Part print with two shaded views. Sizes in mm from the minimum x, y, z corner. A direction names the side the tool comes from. Round coordinates to 2 decimals unless told otherwise and drop trailing zeros. Loops run counter-clockwise (first coordinate to the right, second up) from the corner with the lowest first, then second, coordinate; pieces in that order, holes last. Notation, with made-up numbers: (14.5, 80) - (65.5, 80) arc R19 cw to (65.5, 111) - close; hole circle Ø5 at (67, 62). An arc over 180 degrees is marked (long way). Use a Markdown table: item, result.
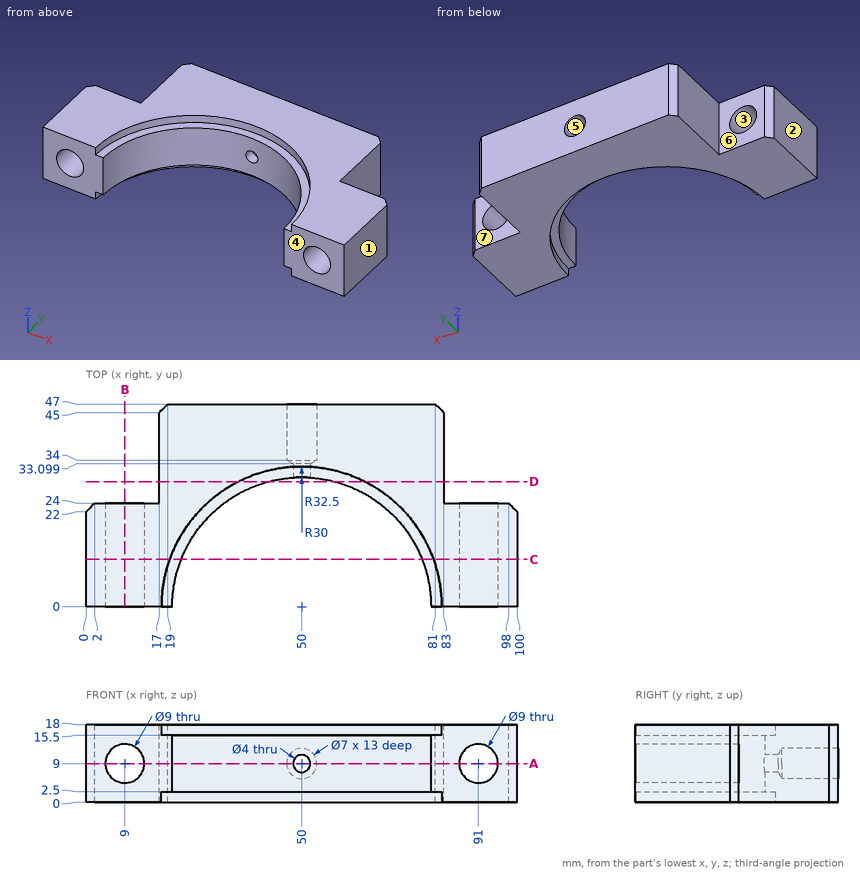
Q1. Which spindle directions (+Z, -Z, +X, -X, +Y, -Y) get a long thin tool onto all of the face, cutting with end or side? Do the marked faces 4, 5, 6 and 7. Say none if no direction does.
Results found:
| item | result |
|---|---|
| face 4 | +Z, -Z, +X, -X, -Y |
| face 5 | +Y |
| face 6 | +Z, -Z, -X, +Y |
| face 7 | +Z, -Z, +X, +Y |
Q2. Cut at C-C, the plane y = 11. List the corners of the cut face in (x, z).
Results found:
| item | result |
|---|---|
| outline | (0, 0) - (19.42, 0) - (19.42, 2.5) - (22.09, 2.5) - (22.09, 15.5) - (19.42, 15.5) - (19.42, 18) - (0, 18) - close; (77.91, 2.5) - (80.58, 2.5) - (80.58, 0) - (100, 0) - (100, 18) - (80.58, 18) - (80.58, 15.5) - (77.91, 15.5) - close; hole circle Ø9 at (9, 9); hole circle Ø9 at (91, 9) |
Q3. Probe line 1 (Z direction, x = 50, y = 41.25); line 2 (X direction, y = 40.75, z = 9); line 3 (Z direction, x = 9, y = 19.25). List the from-to ranges inside material, lowest first.
Results found:
| item | result |
|---|---|
| line 1 | z = 0 to 5.5, 12.5 to 18 |
| line 2 | x = 17 to 46.5, 53.5 to 83 |
| line 3 | z = 0 to 4.5, 13.5 to 18 |
Q4. Cut at A-A, the plane z = 9. Count the separate pieces of the cut face and the enclosed holes in it, plus the area to 3 significant figures.
Results found:
| item | result |
|---|---|
| separate pieces | 4 |
| enclosed holes | 0 |
| area | 1,960 mm2 |
Q5. Cut at B-B, the plane x = 9. List the corners of the cut face in (y, z).
Results found:
| item | result |
|---|---|
| outline | (0, 0) - (24, 0) - (24, 4.5) - (0, 4.5) - close; (0, 13.5) - (24, 13.5) - (24, 18) - (0, 18) - close |
Q6. Pull direction X, two halves, no side cores. Call the marked faces 1, 2 and 3: pulls with the +X half, pulls with the -X half, needs draft (parallel to the pull), parting line crosses it, or undercut.
Results found:
| item | result |
|---|---|
| face 1 | pulls with the +X half |
| face 2 | pulls with the -X half |
| face 3 | undercut |
Q7. Drop flat-ended pins along their axis: pin 1 (16 mm diameter, centred on x = 44, y = 16, fed in from -Z); pin 2 (9 mm diameter, centred on y = 33.5, z = 5.5, fed in from +X); pin 3 (5 mm diameter, centred on x = 50, z = 9, fed in from -Y); pin 4 (6 mm diameter, centred on x = 85.5, z = 13, fed in from +Y). Give the stop position or say it passes through.
Results found:
| item | result |
|---|---|
| pin 1 | passes through |
| pin 2 | stops at x = 83 |
| pin 3 | stops at y = 29.9 |
| pin 4 | stops at y = 45.5 |
Q8. Cut at D-D, the plane y = 29. List the corners of the cut face in (x, z).
Results found:
| item | result |
|---|---|
| outline | (17, 0) - (35.33, 0) - (35.33, 2.5) - (42.32, 2.5) - (42.32, 15.5) - (35.33, 15.5) - (35.33, 18) - (17, 18) - close; (57.68, 2.5) - (64.67, 2.5) - (64.67, 0) - (83, 0) - (83, 18) - (64.67, 18) - (64.67, 15.5) - (57.68, 15.5) - close |
